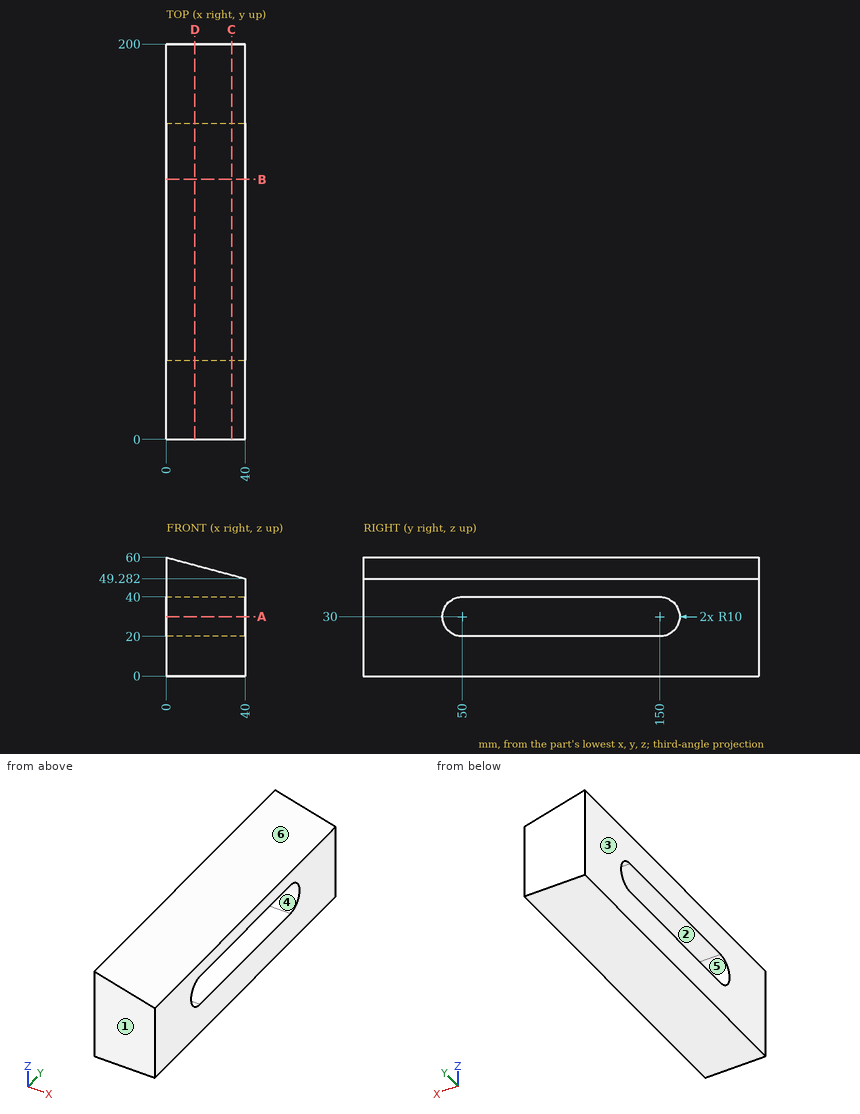
Geometry check sheet. Reference: drawing and pictorial views, mm from the part's lowest x, y, z. A direction names the side the tool comes from. Coordinates: 2 decimals unless noted, no trailing zeros. Order: outer loops, then holes, each group sorted by start corner. A loop starts at its lowest first (then second) coordinate and runs counter-clockwise, first axis right, second up. Notation, with made-up numbers: (60, 85) - (87, 85) arc R19 cw to (87, 89) - close; hole circle Ø10 at (48, 6). An arc over 180 degrees is marked (long way). One line per item, written item: value.
(1) Sectioned sample at C-C (x = 33). Enter the section's corners in (y, z), and give its area (3 significant figures).
Data:
outline: (0, 0) - (200, 0) - (200, 51.16) - (0, 51.16) - close; hole (50, 20) - (150, 20) arc R10 ccw to (150, 40) - (50, 40) arc R10 ccw to start
area: 7,920 mm^2
(2) Sectioned sample at D-D (x = 14.5). Enter the section's corners in (y, z), and give its area (3 significant figures).
Data:
outline: (0, 0) - (200, 0) - (200, 56.11) - (0, 56.11) - close; hole (50, 20) - (150, 20) arc R10 ccw to (150, 40) - (50, 40) arc R10 ccw to start
area: 8,910 mm^2
(3) Depth check by flat-ended pin: pin 1 Ø1.5 at (x, y) = (9.5, 52.5) entering from -Z; pin 2 Ø10 at (y, z) = (115.5, 31) entering from -X. Enter the tip coordinate at first touch or a pass-through.
Data:
pin 1: stops at z = 0
pin 2: passes through
(4) Thickness scan on probe 1 along Z at (x, y) = (34, 92); probe 2 along Z at (x, y) = (27.5, 60); probe 3 along Y at (x, z) = (25, 22). Record the ranges inside material, lowest first. Write a range as from..to.
Data:
probe 1: z = 0..20, 40..50.89
probe 2: z = 0..20, 40..52.63
probe 3: y = 0..44, 156..200
(5) Release check for a two-part mould opening along Z. For the marked faces 3, 4, 5 and 6 record: +Z half, -Z half, draft (parallel to the pull), parting line (faces both ways), or undercut.
Data:
face 3: draft
face 4: undercut
face 5: undercut
face 6: +Z half
(6) Access from +Z, -Z, +X, -X, +Y, -Y to the whole of each face (thin tool, end or side, straight path). Record for the marked faces 1 and 2.
Data:
face 1: +Z, -Z, +X, -X, -Y
face 2: +X, -X
(7) Sectioned sample at A-A (z = 30). Enter the section's corners in (x, y), and give its area (3 significant figures).
Data:
outline: (0, 0) - (40, 0) - (40, 40) - (0, 40) - close; (0, 160) - (40, 160) - (40, 200) - (0, 200) - close
area: 3,200 mm^2
(8) Sectioned sample at B-B (y = 131.5). Enter the section's corners in (x, z), and give its area (3 significant figures).
Data:
outline: (0, 0) - (40, 0) - (40, 20) - (0, 20) - close; (0, 40) - (40, 40) - (40, 49.28) - (0, 60) - close
area: 1,390 mm^2
